The figure shows three views and two pictorial views of one solid part (mm, origin at its lowest corner). Answer the questions. A direction names the side the tool comes from. Coordinates: 2 decimals unless noted, no trailing zeros. Loops run counter-clockwise (first coordinate to the right, second up) from the corner with the lowest first, then second, coordinate; pieces in that order, holes last. Notation, with made-up numbers: (-11.5, -19.5) -> (8.5, -19.5) arc R27 ccw to (8.5, 10.5) -> close; hole circle Ø9 at (76.25, 82.5). An arc over 180 degrees is marked (long way). Use a Markdown table: item, result. Add a question column.
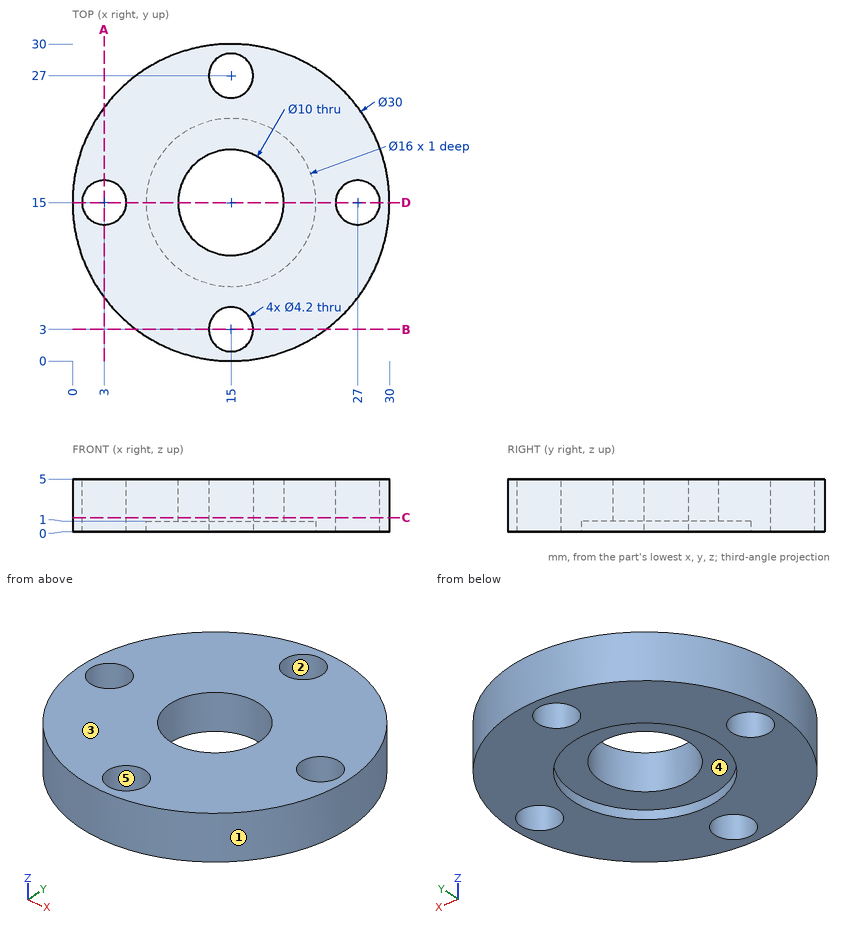
Item 1: For the marked faces 4 and 5, determine the directions among +Z, -Z, +X, -X, +Y, -Y from which every point of the face is accessible in a straight line to the end or side of a thin tool.
Item 2: Section D-D (y = 15) is taken. Determine the outline of the cut face in (x, z).
Item 3: Section C-C (z = 1.35) is taken. Determine the outline of the cut face in (x, y).
Item 4: Given pin 1 (4 mm diameter, centred on x = 15, y = 27, fed in from +Z); pin 2 (14.5 mm diameter, centred on x = 15, y = 15, fed in from -Z); pin 3 (2 mm diameter, centred on x = 9.5, z = 4.5, fed in from +Y); pin 4 (3 mm diameter, centred on y = 10.5, z = 3.5, fed in from +X), each flat-ended and moving along its own axis, determine where each tip first touches the part or whether it passes through.
Item 5: Find the intervals of material crossed by probe 1 along Y at (x, z) = (16.5, 1.65); probe 2 along Y at (x, z) = (15, 1.35); probe 3 along X at (y, z) = (17.75, 0.5), in increasing order.
Item 6: Section A-A (x = 3) is taken. Determine the outline of the cut face in (y, z).
Item 7: For a pull along Y with two mould halves and no side action, classify the marked faces 1, 2 and 3 as +Y half, -Y half, draft (parallel to the pull), parting line (faces both ways), or undercut.
Output:
| question | item | result |
|---|---|---|
| 1 | face 4 | -Z |
| 1 | face 5 | +Z, -Z |
| 2 | outline | (0, 0) -> (0.9, 0) -> (0.9, 5) -> (0, 5) -> close; (5.1, 0) -> (7, 0) -> (7, 1) -> (10, 1) -> (10, 5) -> (5.1, 5) -> close; (20, 1) -> (23, 1) -> (23, 0) -> (24.9, 0) -> (24.9, 5) -> (20, 5) -> close; (29.1, 0) -> (30, 0) -> (30, 5) -> (29.1, 5) -> close |
| 3 | outline | circle Ø30 at (15, 15); hole circle Ø4.2 at (3, 15); hole circle Ø10 at (15, 15); hole circle Ø4.2 at (15, 3); hole circle Ø4.2 at (15, 27); hole circle Ø4.2 at (27, 15) |
| 4 | pin 1 | passes through |
| 4 | pin 2 | stops at z = 1 |
| 4 | pin 3 | stops at y = 29.31 |
| 4 | pin 4 | stops at x = 29.7 |
| 5 | probe 1 | y = 0.08 to 1.53, 4.47 to 10.23, 19.77 to 25.53, 28.47 to 29.92 |
| 5 | probe 2 | y = 0 to 0.9, 5.1 to 10, 20 to 24.9, 29.1 to 30 |
| 5 | probe 3 | x = 0.25 to 7.49, 22.51 to 29.75 |
| 6 | outline | (6, 0) -> (12.9, 0) -> (12.9, 5) -> (6, 5) -> close; (17.1, 0) -> (24, 0) -> (24, 5) -> (17.1, 5) -> close |
| 7 | face 1 | parting line |
| 7 | face 2 | undercut |
| 7 | face 3 | draft |
